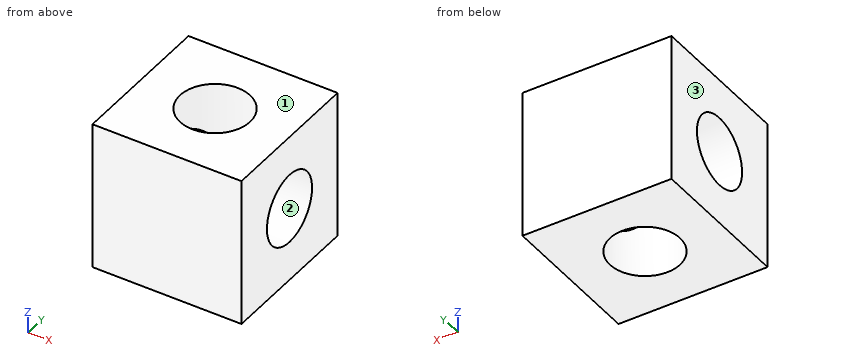
```python
from build123d import *

# Parameters (mm, degrees)
BLOCK_PROFILE_20_32_SQUARE_W = 20.32
BLOCK_PROFILE_20_32_SQUARE_H = 20.32
CUBE_BLOCK_20_32_DEPTH       = 20.32
CROSS_HOLE_A_PROFILE_R       = 4.775
CROSS_HOLE_A_9_35_DEPTH      = 31.48
CROSS_HOLE_B_PROFILE_R       = 4.775
CROSS_HOLE_B_9_35_DEPTH      = 31.48


with BuildPart() as part:
    # Block Profile 20.32 Square → Cube Block 20.32 (new body)
    with BuildSketch(Plane(origin=(0, 0, 0), x_dir=(1, 0, 0), z_dir=(0, 1, 0))):
        Rectangle(BLOCK_PROFILE_20_32_SQUARE_W, BLOCK_PROFILE_20_32_SQUARE_H)
    extrude(amount=CUBE_BLOCK_20_32_DEPTH)

    # Cross Hole A Profile → Cross Hole A Ø9.35 (cut, through all)
    with BuildSketch(Plane.XY.offset(10.16)):
        with Locations((0, 10.16)):
            Circle(CROSS_HOLE_A_PROFILE_R)
    extrude(amount=-CROSS_HOLE_A_9_35_DEPTH, mode=Mode.SUBTRACT)

    # Cross Hole B Profile → Cross Hole B Ø9.35 (cut, through all)
    with BuildSketch(Plane(origin=(10.16, 0, 0), x_dir=(0, 0, -1), z_dir=(1, 0, 0))):
        with Locations((0, 10.16)):
            Circle(CROSS_HOLE_B_PROFILE_R)
    extrude(amount=-CROSS_HOLE_B_9_35_DEPTH, mode=Mode.SUBTRACT)


solid = part.part
```
Geometry: final body of the model. Coordinates: model frame, mm. Face numbers are marked on the shaded views. Round coordinates to 2 decimals unless told otherwise and drop trailing zeros. Write each loop counter-clockwise with the first axis right and the second up, starting at its lowest first coordinate (ties: lowest second). Pieces come first, ordered by that corner, then holes. Notation, with made-up numbers: (60.5, -31) -> (67.5, -31) arc R18 cw to (67.5, -11) -> close; hole circle Ø7 at (57, 83.5). An arc over 180 degrees is marked (long way). Return JSON: item names as keys, results as strings.
Q1. Section A-A on y = 10.16. Return the cut outline in (x, z) (3 decimals).
From the geometry:
{"outline": "(-10.16, -10.16) -> (-4.775, -10.16) -> (-4.775, -4.775) -> (-10.16, -4.775) -> close; (-10.16, 4.775) -> (-4.775, 4.775) -> (-4.775, 10.16) -> (-10.16, 10.16) -> close; (4.775, -10.16) -> (10.16, -10.16) -> (10.16, -4.775) -> (4.775, -4.775) -> close; (4.775, 4.775) -> (10.16, 4.775) -> (10.16, 10.16) -> (4.775, 10.16) -> close"}
Q2. Ray query, line 1 (Y direction, x = 4.5, z = 0) (3 decimals); line 2 (Z direction, x = 6.75, y = 10.16) (3 decimals). Return the intervals inside material, ascending.
From the geometry:
{"line 1": "0 to 5.385, 14.935 to 20.32", "line 2": "-10.16 to -4.775, 4.775 to 10.16"}
Q3. Section C-C on x = 9.25. Return the cut outline in (y, z) (3 decimals).
From the geometry:
{"outline": "(0, -10.16) -> (20.32, -10.16) -> (20.32, 10.16) -> (0, 10.16) -> close; hole circle Ø9.55 at (10.16, 0)"}
Q4. First-contact query: pin 1 Ø8.5 at (x, y) = (0, 10.16) entering from -Z. Flat tip, straight axial feed; report the tip coordinate or a pass-through.
From the geometry:
{"pin 1": "through"}
Q5. Section D-D on x = -2.25. Return the cut outline in (y, z) (3 decimals), and give its area (3 significant figures).
From the geometry:
{"outline": "(0, -10.16) -> (5.948, -10.16) -> (5.948, -2.25) arc R4.775 cw to (5.948, 2.25) -> (5.948, 10.16) -> (0, 10.16) -> close; (14.372, -10.16) -> (20.32, -10.16) -> (20.32, 10.16) -> (14.372, 10.16) -> (14.372, 2.25) arc R4.775 cw to (14.372, -2.25) -> close", "area": "238 mm2"}
Q6. Mould query, pull axis Z, two halves, no side actions, for the marked faces 1, 2 and 3. Classes: +Z half, -Z half, draft (parallel to the pull), parting line (faces both ways), or undercut.
From the geometry:
{"face 1": "+Z half", "face 2": "undercut", "face 3": "draft"}
Q7. Section B-B on z = -3.75. Return the cut outline in (x, y) (3 decimals).
From the geometry:
{"outline": "(-10.16, 0) -> (10.16, 0) -> (10.16, 7.204) -> (3.75, 7.204) arc R4.775 cw to (-3.75, 7.204) -> (-10.16, 7.204) -> close; (-10.16, 13.116) -> (-3.75, 13.116) arc R4.775 cw to (3.75, 13.116) -> (10.16, 13.116) -> (10.16, 20.32) -> (-10.16, 20.32) -> close"}
